from build123d import *

# Parameters (mm, degrees)
SKETCH1_W           = 130
SKETCH1_H           = 130
BOSS_EXTRUDE1_DEPTH = 60
SKETCH2_R           = 15.5
CUT_EXTRUDE1_DEPTH  = 204
SKETCH3_R           = 7.5
CUT_EXTRUDE2_DEPTH  = 40
SKETCH4_R           = 4.1
CUT_EXTRUDE3_DEPTH  = 40
SKETCH5_R           = 6.294295411
SKETCH5_R_2         = 5.5
CUT_EXTRUDE4_DEPTH  = 104


with BuildPart() as part:
    # Sketch1 → Boss-Extrude1 (new body)
    with BuildSketch(Plane(origin=(0, 0, 0), x_dir=(1, 0, 0), z_dir=(0, 1, 0))):
        Rectangle(SKETCH1_W, SKETCH1_H)
    extrude(amount=BOSS_EXTRUDE1_DEPTH)

    # Sketch2 → Cut-Extrude1 (cut)
    with BuildSketch(Plane(origin=(0, 0, -65), x_dir=(-1, 0, 0), z_dir=(0, 0, -1))):
        with Locations((-25, 30)):
            Circle(SKETCH2_R)
        with Locations((25, 30)):
            Circle(SKETCH2_R)
    extrude(amount=-CUT_EXTRUDE1_DEPTH, mode=Mode.SUBTRACT)

    # Sketch3 → Cut-Extrude2 (cut)
    with BuildSketch(Plane(origin=(0, 60, 0), x_dir=(1, 0, 0), z_dir=(0, 1, 0))):
        with Locations(Location((-50, 45, 0), (0, 0, 270))):
            Circle(SKETCH3_R)
        with Locations(Location((50, 45, 0), (0, 0, 270))):
            Circle(SKETCH3_R)
        with Locations(Location((50, -45, 0), (0, 0, 270))):
            Circle(SKETCH3_R)
        with Locations(Location((-50, -45, 0), (0, 0, 270))):
            Circle(SKETCH3_R)
    extrude(amount=-CUT_EXTRUDE2_DEPTH, mode=Mode.SUBTRACT)

    # Sketch4 → Cut-Extrude3 (cut)
    with BuildSketch(Plane(origin=(0, 20, 0), x_dir=(1, 0, 0), z_dir=(0, 1, 0))):
        with Locations(Location((50, 45, 0), (0, 0, 270))):
            Circle(SKETCH4_R)
        with Locations(Location((-50, 45, 0), (0, 0, 270))):
            Circle(SKETCH4_R)
        with Locations(Location((-50, -45, 0), (0, 0, 270))):
            Circle(SKETCH4_R)
        with Locations(Location((50, -45, 0), (0, 0, 270))):
            Circle(SKETCH4_R)
    extrude(amount=-CUT_EXTRUDE3_DEPTH, mode=Mode.SUBTRACT)

    # Sketch5 → Cut-Extrude4 (cut)
    with BuildSketch(Plane(origin=(0, 60, 0), x_dir=(1, 0, 0), z_dir=(0, 1, 0))):
        with Locations(Location((25, 45, 0), (0, 0, 270))):
            Circle(SKETCH5_R)
        with Locations(Location((-25, 45, 0), (0, 0, 270))):
            Circle(SKETCH5_R_2)
    extrude(amount=-CUT_EXTRUDE4_DEPTH, mode=Mode.SUBTRACT)


solid = part.part
CAD build for the part. Positions are in the model's coordinates, mm. A direction names the side the tool comes from. Round coordinates to 2 decimals unless told otherwise and drop trailing zeros. Loops run counter-clockwise (first coordinate to the right, second up) from the corner with the lowest first, then second, coordinate; pieces in that order, holes last.
(1) Cut at A-A (x = -25). Give the cut face in (y, z), plus the area to 3 significant figures.
(2) Two-plate mould, pull along Y, no slides. Class faces 1 (the cylindrical face through (-39.318, 24.063, -0.91)), 2 (the flat face through (46.8, 20, 48.2)), 3 (the flat face through (-65, 30, 1)): +Y half, -Y half, draft (parallel to the pull), parting line (faces both ways), or undercut.
(3) Wall check: line 1 along X through (y, z) = (29.5, -5.5); line 2 along X through (y, z) = (3, -45); line 3 along X through (y, z) = (46, -45). Give the ranges that are in metal, low to high.
(4) Cut at C-C (y = 30). Give the cut face in (x, z), plus the area to 3 significant figures.
(5) Cut at D-D (x = 50). Give the cut face in (y, z), plus the area to 3 significant figures.
(6) Which spindle directions (+Z, -Z, +X, -X, +Y, -Y) get a long thin tool onto all of the face, cutting with end or side? Do faces 4 (the cylindrical face through (43.346, 40.28, 48.461)), 5 (the cylindrical face through (-23.348, 52.354, -39.754)). Say none if no direction does.
(7) Cut at B-B (z = 45). Give the cut face in (x, y).
Findings below:
1. outline: (0, -65) - (14.5, -65) - (14.5, -50.5) - (0, -50.5) - close; (0, -39.5) - (14.5, -39.5) - (14.5, 65) - (0, 65) - close; (45.5, -65) - (60, -65) - (60, -50.5) - (45.5, -50.5) - close; (45.5, -39.5) - (60, -39.5) - (60, 65) - (45.5, 65) - close
1. area: 3,450 mm2
2. face 1: undercut
2. face 2: +Y half
2. face 3: draft
3. line 1: x = -65 to -40.49, -9.51 to 9.51, 40.49 to 65
3. line 2: x = -65 to -54.1, -45.9 to -30.5, -19.5 to 18.71, 31.29 to 45.9, 54.1 to 65
3. line 3: x = -65 to -57.5, -42.5 to -30.5, -19.5 to 18.71, 31.29 to 42.5, 57.5 to 65
4. outline: (-65, -65) - (-40.5, -65) - (-40.5, 65) - (-65, 65) - close; (-9.5, -65) - (9.5, -65) - (9.5, 65) - (-9.5, 65) - close; (40.5, -65) - (65, -65) - (65, 65) - (40.5, 65) - close; hole circle Ø15 at (-50, -45); hole circle Ø15 at (-50, 45); hole circle Ø15 at (50, -45); hole circle Ø15 at (50, 45)
4. area: 8,130 mm2
5. outline: (0, -65) - (60, -65) - (60, -52.5) - (20, -52.5) - (20, -49.1) - (0, -49.1) - close; (0, -40.9) - (20, -40.9) - (20, -37.5) - (60, -37.5) - (60, 37.5) - (20, 37.5) - (20, 40.9) - (0, 40.9) - close; (0, 49.1) - (20, 49.1) - (20, 52.5) - (60, 52.5) - (60, 65) - (0, 65) - close
5. area: 6,270 mm2
6. face 4: +Y
6. face 5: +Y, -Y
7. outline: (-65, 0) - (-54.1, 0) - (-54.1, 20) - (-57.5, 20) - (-57.5, 60) - (-65, 60) - close; (-45.9, 0) - (45.9, 0) - (45.9, 20) - (42.5, 20) - (42.5, 60) - (-42.5, 60) - (-42.5, 20) - (-45.9, 20) - close; (54.1, 0) - (65, 0) - (65, 60) - (57.5, 60) - (57.5, 20) - (54.1, 20) - close; hole circle Ø31 at (-25, 30); hole circle Ø31 at (25, 30)
